```python
from build123d import *

# Parameters (mm, degrees)
BOSS_EXTRUDE1_DEPTH = 7.5


with BuildPart() as part:
    # Sketch1 → Boss-Extrude1 (new, symmetric)
    with BuildSketch(Plane(origin=(0, 0, 0), x_dir=(0, 0, -1), z_dir=(1, 0, 0))):
        Polygon((0, 0), (0, 125), (-80, 125), (-80, 95), (-20, 0), align=None)
    extrude(amount=BOSS_EXTRUDE1_DEPTH, both=True)


solid = part.part
```
Read the model definition and answer for the solid it produces. Units are mm, in the model's axes. Give positions to 0.01 mm unless a question says otherwise; leave off trailing zeros. Write each loop counter-clockwise with the first axis right and the second up, starting at its lowest first coordinate (ties: lowest second). Pieces come first, ordered by that corner, then holes. Notation, with made-up numbers: (-7.75, 7) -> (17.25, 7) arc R21 cw to (17.25, 42) -> close; hole circle Ø3 at (36, 25.25). An arc over 180 degrees is marked (long way). Answer in a Markdown table with one row per item.
1) Straight lines are drawn through the part: line 1 (Z direction, x = -2, y = 35); line 2 (Y direction, x = 3.25, z = 65); line 3 (Y direction, x = -4.5, z = 67.5). For each, find the intervals that lie inside material, in ascending order. Write a range as [from, to].
Results list:
| item | result |
|---|---|
| line 1 | [0, 42.11] |
| line 2 | [71.25, 125] |
| line 3 | [75.21, 125] |
2) Section C-C on y = 20 is taken. Give the vertices of the cut face in (x, z).
Results list:
| item | result |
|---|---|
| outline | (-7.5, 0) -> (7.5, 0) -> (7.5, 32.63) -> (-7.5, 32.63) -> close |
3) Section A-A on x = -1.75 is taken. Give the vertices of the cut face in (y, z), plus the area to 3 significant figures.
Results list:
| item | result |
|---|---|
| outline | (0, 0) -> (125, 0) -> (125, 80) -> (95, 80) -> (0, 20) -> close |
| area | 7,150 mm^2 |
4) Section B-B on z = 74 is taken. Give the vertices of the cut face in (x, y), plus the area to 4 significant figures.
Results list:
| item | result |
|---|---|
| outline | (-7.5, 85.5) -> (7.5, 85.5) -> (7.5, 125) -> (-7.5, 125) -> close |
| area | 592.5 mm^2 |
5) Each of these flat-tipped pins is pushed along its axis until it touches: pin 1 Ø2 at (x, y) = (-2, 70.5) entering from +Z; pin 2 Ø1.5 at (x, y) = (2, 60) entering from +Z; pin 3 Ø1 at (x, y) = (-2.5, 46) entering from +Z. Where does it stop, or does it pass through?
Results list:
| item | result |
|---|---|
| pin 1 | z = 65.16 |
| pin 2 | z = 58.37 |
| pin 3 | z = 49.37 |
